Drawing for the job (mm, zero at the part's lowest x, y, z). A direction names the side the tool comes from. Round coordinates to 2 decimals unless told otherwise and drop trailing zeros. Order: outer loops, then holes, each group sorted by start corner. A loop starts at its lowest first (then second) coordinate and runs counter-clockwise, first axis right, second up. Notation, with made-up numbers: (84, 32.5) - (128, 32.5) arc R11 cw to (128, 42.5) - close; hole circle Ø3 at (10.25, 1.25). An arc over 180 degrees is marked (long way). Answer as a JSON object with one key per item and string values.
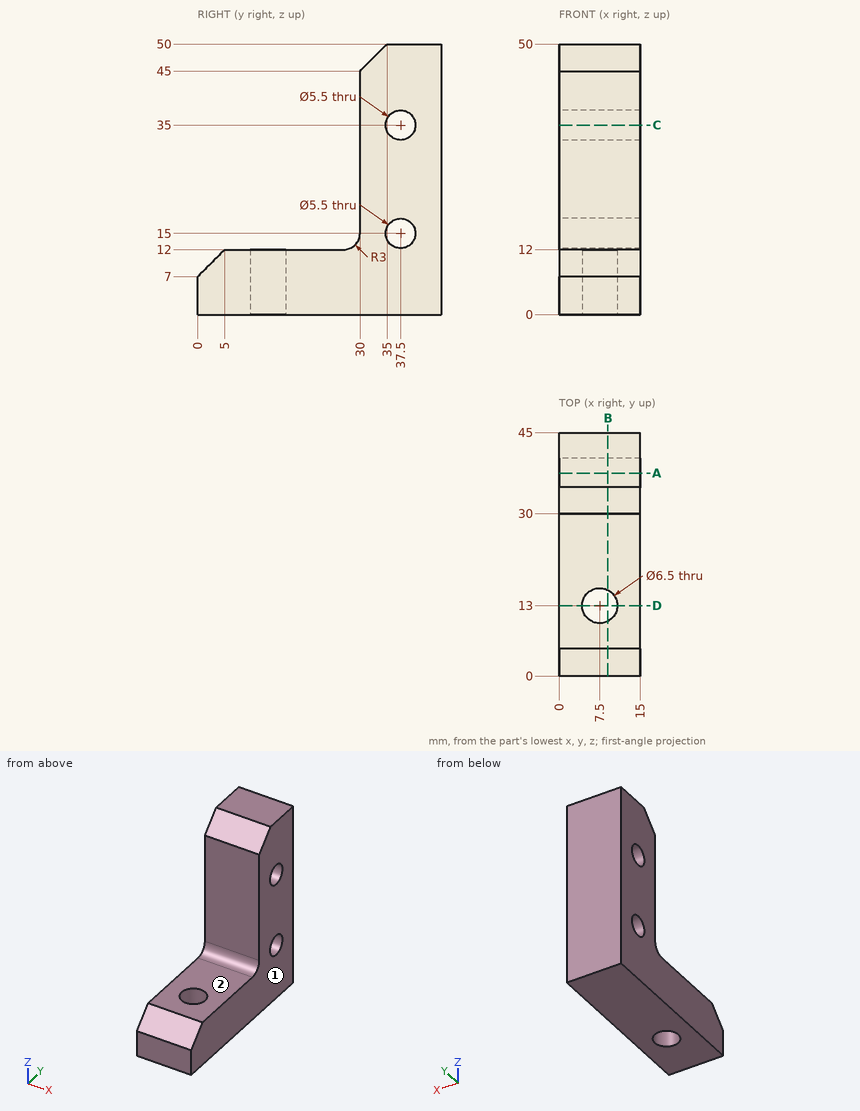
Item 1: Cut at B-B (x = 9). Write the cut outline in (y, z), plus the area to 3 significant figures.
Taken from the geometry:
{"outline": "(0, 0) - (10.12, 0) - (10.12, 12) - (5, 12) - (0, 7) - close; (15.88, 0) - (45, 0) - (45, 50) - (35, 50) - (30, 45) - (30, 15) arc R3 cw to (27, 12) - (15.88, 12) - close; hole circle Ø5.5 at (37.5, 15); hole circle Ø5.5 at (37.5, 35)", "area": "970 mm2"}
Item 2: Cut at C-C (z = 35). Write the cut outline in (x, y), plus the area to 4 significant figures.
Taken from the geometry:
{"outline": "(0, 30) - (15, 30) - (15, 34.75) - (0, 34.75) - close; (0, 40.25) - (15, 40.25) - (15, 45) - (0, 45) - close", "area": "142.5 mm2"}
Item 3: Tool access for the marked faces 1 and 2: list every direction of +Z, -Z, +X, -X, +Y, -Y with a clear straight run to the whole face (end or side of a thin tool).
Taken from the geometry:
{"face 1": "+Z, -Z, +X, +Y, -Y", "face 2": "+Z, +X, -X, -Y"}
Item 4: Drop flat-ended pins along their axis: P1, Ø5, axis at y = 28.5, z = 14, coming from the -X side; P2, Ø4.5, axis at x = 11, y = 17, coming from the +Z side; P3, Ø4.5, axis at x = 5.5, z = 29.5, coming from the -Y side; P4, Ø4, axis at x = 7.5, y = 13, coming from the +Z side. Give the stop position or say it passes through.
Taken from the geometry:
{"P1": "x = 0", "P2": "z = 12", "P3": "y = 30", "P4": "through"}
Item 5: Probe L1, parallel to Y at x = 7.5, z = 6; L2, parallel to Y at x = 9, z = 15; L3, parallel to Z at x = 2.5, y = 8.5. List the from-to ranges inside material, lowest first. Write a range as from..to.
Taken from the geometry:
{"L1": "0..9.75, 16.25..45", "L2": "30..34.75, 40.25..45", "L3": "0..12"}
Item 6: Cut at A-A (y = 37.5). Write the cut outline in (x, z), plus the area to 3 significant figures.
Taken from the geometry:
{"outline": "(0, 0) - (15, 0) - (15, 12.25) - (0, 12.25) - close; (0, 17.75) - (15, 17.75) - (15, 32.25) - (0, 32.25) - close; (0, 37.75) - (15, 37.75) - (15, 50) - (0, 50) - close", "area": "585 mm2"}
Item 7: Cut at D-D (y = 13). Write the cut outline in (x, z).
Taken from the geometry:
{"outline": "(0, 0) - (4.25, 0) - (4.25, 12) - (0, 12) - close; (10.75, 0) - (15, 0) - (15, 12) - (10.75, 12) - close"}
